Source: CAD feature listing. Evaluate the final solid. Frame: model axes, mm. Coordinates: 2 decimals unless noted, no trailing zeros. Order: outer loops, then holes, each group sorted by start corner. A loop starts at its lowest first (then second) coordinate and runs counter-clockwise, first axis right, second up. Notation, with made-up numbers: (-19.5, 5) -> (17.5, 5) arc R21 cw to (17.5, 14) -> close; hole circle Ø8 at (17.5, 62.25). An arc over 180 degrees is marked (long way). Put each result on its own line as item: value.
from build123d import *

# Parameters (mm, degrees)
SKETCH1_W                  = 230
SKETCH1_H                  = 200
BOSS_EXTRUDE1_DEPTH        = 6
M5_TAPPED_HOLE1_AT_2_COUNT = 2
M5_TAPPED_HOLE1_AT_2_PITCH = 109
M5_TAPPED_HOLE1_AT_3_COUNT = 2
M5_TAPPED_HOLE1_AT_3_PITCH = 218


with BuildPart() as part:
    # Sketch1 → Boss-Extrude1 (new, symmetric)
    with BuildSketch(Plane(origin=(0, 0, 0), x_dir=(0, 0, -1), z_dir=(1, 0, 0))):
        Rectangle(SKETCH1_W, SKETCH1_H)
    extrude(amount=BOSS_EXTRUDE1_DEPTH, both=True)

    # Sketch3 → M5 Tapped Hole1 (revolve, cut)
    with BuildSketch(Plane(origin=(0, 100, -109), x_dir=(0, 0, 1), z_dir=(1, 0, 0))):
        Polygon((0, 0), (0, 25.7618073), (2.1, 24.5), (2.1, 0), align=None)
    m5_tapped_hole1 = revolve(axis=Axis((0, 106.35, -109), (0, -1, 0)), mode=Mode.SUBTRACT)

    # M5 Tapped Hole1 at 2: M5 Tapped Hole1 ×2
    with Locations(*[(0, 0, i * M5_TAPPED_HOLE1_AT_2_PITCH) for i in range(1, M5_TAPPED_HOLE1_AT_2_COUNT)]):
        add(m5_tapped_hole1, mode=Mode.SUBTRACT)

    # M5 Tapped Hole1 at 3: M5 Tapped Hole1 ×2
    with Locations(*[(0, 0, i * M5_TAPPED_HOLE1_AT_3_PITCH) for i in range(1, M5_TAPPED_HOLE1_AT_3_COUNT)]):
        add(m5_tapped_hole1, mode=Mode.SUBTRACT)

    # Mirror1: M5 Tapped Hole1 across plane
    add(m5_tapped_hole1.mirror(Plane.ZX), mode=Mode.SUBTRACT)

    # Mirror1 copy 1 sketch → Mirror1 copy 1 (revolve, cut)
    with BuildSketch(Plane(origin=(0, -100, 0), x_dir=(0, 0, 1), z_dir=(1, 0, 0))):
        Polygon((0, 0), (0, -25.7618073), (2.1, -24.5), (2.1, 0), align=None)
    revolve(axis=Axis((0, -106.35, 0), (0, -1, 0)), mode=Mode.SUBTRACT)

    # Mirror1 copy 2 sketch → Mirror1 copy 2 (revolve, cut)
    with BuildSketch(Plane(origin=(0, -100, 109), x_dir=(0, 0, 1), z_dir=(1, 0, 0))):
        Polygon((0, 0), (0, -25.7618073), (2.1, -24.5), (2.1, 0), align=None)
    revolve(axis=Axis((0, -106.35, 109), (0, -1, 0)), mode=Mode.SUBTRACT)


solid = part.part
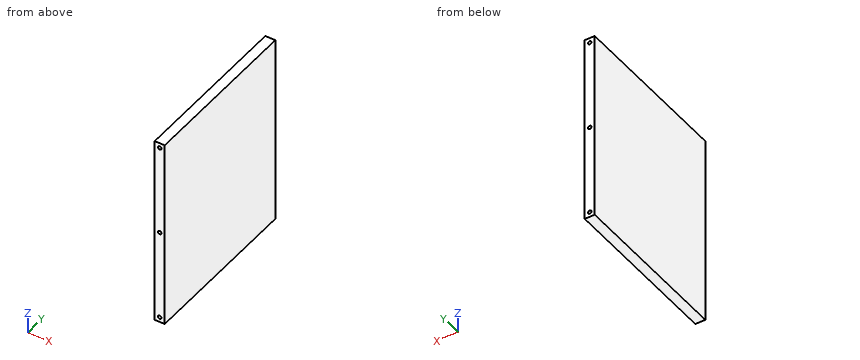
1. Ray query, line 1 along Z through (x, y) = (0, 83.75); line 2 along X through (y, z) = (81.5, 109). Return the intervals inside material, ascending.
Numbers:
line 1: z = -115 to -111.1, -106.9 to -2.1, 2.1 to 106.9, 111.1 to 115
line 2: x = -6 to -2.1, 2.1 to 6
2. First-contact query: pin 1 (6.5 mm diameter, centred on x = 0, z = -109, fed in from -Y); pin 2 (3.5 mm diameter, centred on x = 0, z = 0, fed in from -Y); pin 3 (3.5 mm diameter, centred on x = 0, z = -109, fed in from +Y); pin 4 (4 mm diameter, centred on x = 0, z = 0, fed in from +Y). Flat tips, straight axial feed; report the tip coordinate or a pass-through.
Numbers:
pin 1: stops at y = -100
pin 2: stops at y = -75.29
pin 3: stops at y = 75.29
pin 4: stops at y = 75.44
3. Cut plane A-A on y = 81. Output: boundary loops of the cut face in (x, z).
Numbers:
outline: (-6, -115) -> (6, -115) -> (6, 115) -> (-6, 115) -> close; hole circle Ø4.2 at (0, -109); hole circle Ø4.2 at (0, 0); hole circle Ø4.2 at (0, 109)
